Part model, mm, in its own coordinate system. A direction names the side the tool comes from. Give positions to 0.01 mm unless a question says otherwise; leave off trailing zeros. Order: outer loops, then holes, each group sorted by start corner. A loop starts at its lowest first (then second) coordinate and runs counter-clockwise, first axis right, second up.
from build123d import *

# Parameters (mm, degrees)
SKETCH1_W           = 32
SKETCH1_H           = 45
BOSS_EXTRUDE1_DEPTH = 8
M12_TAPPED_HOLE1_D  = 10.2
CUT_EXTRUDE1_DEPTH  = 29.744564704
CUT_EXTRUDE2_DEPTH  = 3.3
FILLET1_R           = 3


with BuildPart() as part:
    # Sketch1 → Boss-Extrude1 (new body)
    with BuildSketch(Plane.XY):
        Rectangle(SKETCH1_W, SKETCH1_H)
    extrude(amount=BOSS_EXTRUDE1_DEPTH)

    # M12 Tapped Hole1 (through all)
    with Locations(Plane.XY.offset(8)):
        with Locations((0, 0)):
            Hole(M12_TAPPED_HOLE1_D / 2)

    # Sketch5 → Cut-Extrude1 (cut, through all)
    with BuildSketch(Plane.XY.offset(8)):
        with BuildLine():
            Line((-5, -12.75), (5, -12.75))
            ThreePointArc((5, -12.75), (6.75, -14.5), (5, -16.25))
            Line((5, -16.25), (-5, -16.25))
            ThreePointArc((-5, -16.25), (-6.75, -14.5), (-5, -12.75))
        make_face()
        with BuildLine():
            Line((-5, 16.25), (5, 16.25))
            ThreePointArc((5, 16.25), (6.75, 14.5), (5, 12.75))
            Line((5, 12.75), (-5, 12.75))
            ThreePointArc((-5, 12.75), (-6.75, 14.5), (-5, 16.25))
        make_face()
    extrude(amount=-CUT_EXTRUDE1_DEPTH, mode=Mode.SUBTRACT)

    # Sketch6 → Cut-Extrude2 (cut)
    with BuildSketch(Plane.XY.offset(8)):
        with BuildLine():
            Line((-5, -11.5), (5, -11.5))
            ThreePointArc((5, -11.5), (8, -14.5), (5, -17.5))
            Line((5, -17.5), (-5, -17.5))
            ThreePointArc((-5, -17.5), (-8, -14.5), (-5, -11.5))
        make_face()
        with BuildLine():
            Line((-5, 17.5), (5, 17.5))
            ThreePointArc((5, 17.5), (8, 14.5), (5, 11.5))
            Line((5, 11.5), (-5, 11.5))
            ThreePointArc((-5, 11.5), (-8, 14.5), (-5, 17.5))
        make_face()
    extrude(amount=-CUT_EXTRUDE2_DEPTH, mode=Mode.SUBTRACT)

    # Fillet1
    fillet1_edges = [part.edges().sort_by_distance(p)[0] for p in [
        (-16, 22.5, 4),
        (16, 22.5, 4),
        (16, -22.5, 4),
        (-16, -22.5, 4),
    ]]
    fillet(fillet1_edges, radius=FILLET1_R)


solid = part.part
Item 1: Band-saw the part on A-A on y = 14.5. List the corners of the cut face in (x, z), plus the area to 3 significant figures.
Item 2: Band-saw the part on B-B on z = 7. List the corners of the cut face in (x, y), plus the area to 3 significant figures.
Item 3: Which spindle directions (+Z, -Z, +X, -X, +Y, -Y) get a long thin tool onto all of the face, cutting with end or side? Do faces 1 (the face through (-15.14, -21.6, 4.06)), 2 (the face through (-8, 14.4, 6.4)), 3 (the face through (6.75, 14.54, 2.38)). Say none if no direction does.
Item 4: Drop flat-ended pins along their axis: P1, Ø6, axis at x = 4, y = 2, coming from the +Z side; P2, Ø1.8, axis at x = -2.5, y = 13.5, coming from the +Z side. Give the stop position or say it passes through.
Item 5: Pull direction Y, two halves, no side cores. Call faces 4 (the face through (0, -16.25, 2)), 5 (the face through (15.1, -21.64, 4.06)), 6 (the face through (-16, 0, 4)), 7 (the face through (0.1, 12.5, 4.7)): released by +Y, released by -Y, zero draft, split by the parting line, or undercut.
Item 6: Band-saw the part on C-C on x = 0. List the corners of the cut face in (y, z), plus the area to 3 significant figures.
Item 7: Band-saw the part on D-D on y = 0. List the corners of the cut face in (x, z), plus the area to 3 significant figures.
Item 8: Drill centre lines: probe 1 along Y at (x, z) = (0, 5.5); probe 2 along Y at (x, z) = (0, 1.5); probe 3 along Y at (x, z) = (6, 4.75). Where is each one in solid material? Low to high.
Working result:
1. outline: (-16, 0) - (-6.75, 0) - (-6.75, 4.7) - (-8, 4.7) - (-8, 8) - (-16, 8) - close; (6.75, 0) - (16, 0) - (16, 8) - (8, 8) - (8, 4.7) - (6.75, 4.7) - close
1. area: 140 mm2
2. outline: (-16, -19.5) arc R3 ccw to (-13, -22.5) - (13, -22.5) arc R3 ccw to (16, -19.5) - (16, 19.5) arc R3 ccw to (13, 22.5) - (-13, 22.5) arc R3 ccw to (-16, 19.5) - close; hole circle Ø10.2 at (0, 0); hole (-5, -17.5) - (5, -17.5) arc R3 ccw to (5, -11.5) - (-5, -11.5) arc R3 ccw to start; hole (-5, 11.5) - (5, 11.5) arc R3 ccw to (5, 17.5) - (-5, 17.5) arc R3 ccw to start
2. area: 1,170 mm2
3. face 1: +Z, -Z, -X, -Y
3. face 2: +Z
3. face 3: +Z, -Z
4. P1: stops at z = 8
4. P2: stops at z = 4.7
5. face 4: undercut
5. face 5: released by -Y
5. face 6: zero draft
5. face 7: undercut
6. outline: (-22.5, 0) - (-16.25, 0) - (-16.25, 4.7) - (-17.5, 4.7) - (-17.5, 8) - (-22.5, 8) - close; (-12.75, 0) - (-5.1, 0) - (-5.1, 8) - (-11.5, 8) - (-11.5, 4.7) - (-12.75, 4.7) - close; (5.1, 0) - (12.75, 0) - (12.75, 4.7) - (11.5, 4.7) - (11.5, 8) - (5.1, 8) - close; (16.25, 0) - (22.5, 0) - (22.5, 8) - (17.5, 8) - (17.5, 4.7) - (16.25, 4.7) - close
6. area: 206 mm2
7. outline: (-16, 0) - (-5.1, 0) - (-5.1, 8) - (-16, 8) - close; (5.1, 0) - (16, 0) - (16, 8) - (5.1, 8) - close
7. area: 174 mm2
8. probe 1: y = -22.5 to -17.5, -11.5 to -5.1, 5.1 to 11.5, 17.5 to 22.5
8. probe 2: y = -22.5 to -16.25, -12.75 to -5.1, 5.1 to 12.75, 16.25 to 22.5
8. probe 3: y = -22.5 to -17.33, -11.67 to 11.67, 17.33 to 22.5
